```python
from build123d import *

# Parameters (mm, degrees)
HUB_PROFILE_SKETCH_R       = 22.5
HUB_PROFILE_SKETCH_R_2     = 10
HUB_BOSS_45_DEPTH          = 30
HUB_START                  = -5
HUB_FACE_SLOT_15_DEPTH     = 5
HUB_SLOT_STEP_15_DEPTH     = 5
CRANK_ARM_PROFILE_SKETCH_W = 20
CRANK_ARM_PROFILE_SKETCH_H = 35
CRANK_ARM_DEPTH            = 80
BORE_START                 = -80
BORE_SKETCH_R              = 10
BORE_20_DEPTH              = 80
ARM_WINDOW_SKETCH_W        = 10
ARM_WINDOW_SKETCH_H        = 20
ARM_WINDOW_10X20_DEPTH     = 50
ARM_SIDE_CUT_SKETCH_R      = 4.5
ARM_SIDE_CUT_DEPTH         = 86.476604986


with BuildPart() as part:
    # Hub Profile Sketch → Hub Boss Ø45 (new body)
    with BuildSketch(Plane(origin=(0, 0, 0), x_dir=(0, 0, -1), z_dir=(1, 0, 0))):
        Circle(HUB_PROFILE_SKETCH_R)
        Circle(HUB_PROFILE_SKETCH_R_2, mode=Mode.SUBTRACT)
    extrude(amount=HUB_BOSS_45_DEPTH)

    # Hub Face Slot Sketch → Hub Face Slot 15 (cut)
    with BuildSketch(Plane(origin=(30, 0, 0), x_dir=(0, 0, -1), z_dir=(1, 0, 0)).offset(HUB_START)):
        with BuildLine():
            Line((-21.213203436, 7.5), (21.213203436, 7.5))
            ThreePointArc((21.213203436, 7.5), (0, 22.5), (-21.213203436, 7.5))
        make_face()
    extrude(amount=HUB_FACE_SLOT_15_DEPTH, mode=Mode.SUBTRACT)

    # Hub Slot Step Sketch → Hub Slot Step 15 (cut)
    with BuildSketch(Plane(origin=(30, 0, 0), x_dir=(0, 0, -1), z_dir=(1, 0, 0)).offset(HUB_START)):
        with BuildLine():
            Line((-21.213203436, -7.5), (21.213203436, -7.5))
            ThreePointArc((21.213203436, -7.5), (0, -22.5), (-21.213203436, -7.5))
        make_face()
    extrude(amount=HUB_SLOT_STEP_15_DEPTH, mode=Mode.SUBTRACT)

    # Crank Arm Profile Sketch → Crank Arm (add)
    with BuildSketch(Plane.XY):
        with Locations((10, 0)):
            Rectangle(CRANK_ARM_PROFILE_SKETCH_W, CRANK_ARM_PROFILE_SKETCH_H)
    extrude(amount=CRANK_ARM_DEPTH)

    # Bore Sketch → Bore Ø20 (cut)
    with BuildSketch(Plane(origin=(20, 0, 0), x_dir=(0, 0, -1), z_dir=(1, 0, 0)).offset(BORE_START)):
        with Locations(Location((0, 0, 0), (0, 0, 131.409622109))):
            Circle(BORE_SKETCH_R)
    extrude(amount=BORE_20_DEPTH, mode=Mode.SUBTRACT)

    # Arm Window Sketch → Arm Window 10x20 (cut)
    with BuildSketch(Plane.XY.offset(80)):
        with Locations((15, 0)):
            Rectangle(ARM_WINDOW_SKETCH_W, ARM_WINDOW_SKETCH_H)
    extrude(amount=-ARM_WINDOW_10X20_DEPTH, mode=Mode.SUBTRACT)

    # Arm Side Cut Sketch → Arm Side Cut (cut, through all)
    with BuildSketch(Plane(origin=(10, 0, 0), x_dir=(0, 0, -1), z_dir=(1, 0, 0))):
        with Locations((-65, 0)):
            Circle(ARM_SIDE_CUT_SKETCH_R)
        with Locations((-45, 0)):
            Circle(ARM_SIDE_CUT_SKETCH_R)
    extrude(amount=-ARM_SIDE_CUT_DEPTH, mode=Mode.SUBTRACT)


solid = part.part
```
The model under review builds one solid part; all positions refer to its coordinate system, in mm. A direction names the side the tool comes from. Give positions to 0.01 mm unless a question says otherwise; leave off trailing zeros. Loops run counter-clockwise (first coordinate to the right, second up) from the corner with the lowest first, then second, coordinate; pieces in that order, holes last. Notation, with made-up numbers: (-38, 66.25) - (-25, 66.25) arc R20 cw to (-25, 86.25) - close; hole circle Ø4 at (-37, 87). An arc over 180 degrees is marked (long way). Answer as a JSON object with one key per item and string values.
Q1. For faces 1 (the flat face through (27, 7.5, 14)), 2 (the flat face through (10, 17.5, 47)), 3 (the flat face through (10, -17.5, 47)), 4 (the flat face through (25, -13, 0)), 5 (the flat face through (10, 0, 55)), list the 3-axis set-ups (+Z, -Z, +X, -X, +Y, -Y) from which the entire face can be reached by the end or side of a thin tool; tool diameter is ignored.
Worked out:
{"face 1": "+Z, -Z, +X, +Y", "face 2": "+Z, +X, -X, +Y", "face 3": "+Z, +X, -X, -Y", "face 4": "+Z, -Z, +X, -Y", "face 5": "+Z, +X"}
Q2. Add section D-D on z = 11.5. State the section outline as (x, y) points, plus the area to 3 significant figures.
Worked out:
{"outline": "(0, -19.34) - (25, -19.34) - (25, -7.5) - (30, -7.5) - (30, 7.5) - (25, 7.5) - (25, 19.34) - (0, 19.34) - close", "area": "1,040 mm^2"}
Q3. Insertion check: pin 1 (2 mm diameter, centred on x = 17.5, z = 51.5, fed in from +Y); pin 2 (2 mm diameter, centred on x = 19, y = -2, fed in from -Z); pin 3 (3 mm diameter, centred on x = 14.5, z = 46, fed in from -Y); pin 4 (11.5 mm diameter, centred on y = 0, z = 65, fed in from -X). Each pin has a flat end and moves straight along its axis. Give the tip position at first contact, or say it passes through.
Worked out:
{"pin 1": "stops at y = 17.5", "pin 2": "stops at z = -22.48", "pin 3": "stops at y = -17.5", "pin 4": "stops at x = 0"}
Q4. Add section A-A on z = 45. State the section outline as (x, y) points.
Worked out:
{"outline": "(0, -17.5) - (20, -17.5) - (20, -10) - (10, -10) - (10, -4.5) - (0, -4.5) - close; (0, 4.5) - (10, 4.5) - (10, 10) - (20, 10) - (20, 17.5) - (0, 17.5) - close"}
Q5. Add section B-B on y = 0. State the section outline as (x, z) points.
Worked out:
{"outline": "(0, -22.5) - (30, -22.5) - (30, -10) - (0, -10) - close; (0, 10) - (30, 10) - (30, 22.5) - (20, 22.5) - (20, 30) - (10, 30) - (10, 40.5) - (0, 40.5) - close; (0, 49.5) - (10, 49.5) - (10, 60.5) - (0, 60.5) - close; (0, 69.5) - (10, 69.5) - (10, 80) - (0, 80) - close"}
Q6. Mouldability with a two-part tool opening along Y and no side actions: class faces 6 (the cylindrical face through (14.79, 6.76, -21.46)), 7 (the flat face through (15, -10, 55)), 8 (the flat face through (20, -12, 47)) as +Y half, -Y half, draft (parallel to the pull), parting line (faces both ways), or undercut.
Worked out:
{"face 6": "parting line", "face 7": "undercut", "face 8": "draft"}
Q7. Add section C-C on x = 21. State the section outline as (y, z) points.
Worked out:
{"outline": "circle Ø45 at (0, 0); hole circle Ø20 at (0, 0)"}
Q8. To check wall thickness, follow line 1 along Y through (x, z) = (13.25, 65); line 2 along Z through (x, y) = (5.5, -1); line 3 along Y through (x, z) = (4.25, 45). State the ranges of each line that lie inside material, in increasing order.
Worked out:
{"line 1": "y = -17.5 to -10, 10 to 17.5", "line 2": "z = -22.48 to -9.95, 9.95 to 40.61, 49.39 to 60.61, 69.39 to 80", "line 3": "y = -17.5 to -4.5, 4.5 to 17.5"}
